```python
from build123d import *

# Parameters (mm, degrees)
BOSS_EXTRUDE1_DEPTH = 32
SKETCH2_R           = 1.75
CUT_EXTRUDE1_DEPTH  = 10
SKETCH3_W           = 67.397349656
SKETCH3_H           = 25.662976956
CUT_EXTRUDE2_DEPTH  = 38.656340887
SKETCH4_R           = 1.75
CUT_EXTRUDE3_DEPTH  = 10


with BuildPart() as part:
    # Sketch1 → Boss-Extrude1 (new body)
    with BuildSketch(Plane(origin=(0, 0, 0), x_dir=(1, 0, 0), z_dir=(0, 1, 0))):
        with BuildLine():
            Line((-8, -10), (-8, -12))
            ThreePointArc((-8, -12), (-8.878679656, -14.121320344), (-11, -15))
            Line((-11, -15), (-13, -15))
            Line((-13, -15), (-13, 15))
            Line((-13, 15), (-1, 15))
            Line((-1, 15), (13, 0))
            Line((13, 0), (13, -15))
            Line((13, -15), (11, -15))
            ThreePointArc((11, -15), (8.878679656, -14.121320344), (8, -12))
            Line((8, -12), (8, -10))
            ThreePointArc((8, -10), (0, -2), (-8, -10))
        make_face()
    extrude(amount=BOSS_EXTRUDE1_DEPTH)

    # Sketch2 → Cut-Extrude1 (cut)
    with BuildSketch(Plane(origin=(13, 0, 0), x_dir=(0, 0, -1), z_dir=(1, 0, 0))):
        with Locations((-10, 26)):
            Circle(SKETCH2_R)
        with Locations((-10, 6)):
            Circle(SKETCH2_R)
    extrude(amount=-CUT_EXTRUDE1_DEPTH, mode=Mode.SUBTRACT)

    # Sketch3 → Cut-Extrude2 (cut, through all)
    with BuildSketch(Plane(origin=(0, 32, 0), x_dir=(1, 0, 0), z_dir=(0, 1, 0))):
        with Locations((-9.275193266, 15.831488478)):
            Rectangle(SKETCH3_W, SKETCH3_H)
    extrude(amount=-CUT_EXTRUDE2_DEPTH, mode=Mode.SUBTRACT)

    # Sketch4 → Cut-Extrude3 (cut)
    with BuildSketch(Plane.ZY.offset(13)):
        with Locations((0, 6)):
            Circle(SKETCH4_R)
        with Locations((0, 26)):
            Circle(SKETCH4_R)
    extrude(amount=-CUT_EXTRUDE3_DEPTH, mode=Mode.SUBTRACT)


solid = part.part
```
Read the model definition and answer for the solid it produces. Units are mm, in the model's axes. A direction names the side the tool comes from. Round coordinates to 2 decimals unless told otherwise and drop trailing zeros. Write each loop counter-clockwise with the first axis right and the second up, starting at its lowest first coordinate (ties: lowest second). Pieces come first, ordered by that corner, then holes. Notation, with made-up numbers: (87.25, 24.25) -> (104.25, 24.25) arc R23 cw to (104.25, 46.25) -> close; hole circle Ø11 at (33.5, -4). An arc over 180 degrees is marked (long way). Answer in a Markdown table with one row per item. Add a question column.
1) Find section B-B, the plane z = 11. Determine the outline of the cut face in (x, y).
2) Find section C-C, the plane y = 15.5. Determine the outline of the cut face in (x, z), and give its area (3 significant figures).
3) Find section A-A, the plane y = 6. Determine the outline of the cut face in (x, z).
4) Which of the six approach directions +Z, -Z, +X, -X, +Y, -Y give full straight-line access (tool end or side, diameter ignored) to faces 1 (the face through (-8.07, 27.735, -0.228)), 2 (the face through (8.9, 15.78, 14.14)), 3 (the face through (10.439, 27.735, 10.228))?
5) Given P1, Ø5, axis at x = 1.5, y = 10.5, coming from the +Z side; P2, Ø3, axis at y = 6, z = 10, coming from the +X side; P3, Ø1, axis at y = 26, z = -1, coming from the -X side, each flat-ended and moving along its own axis, determine where each tip first touches the part or whether it passes through.
6) Determine the mould class of faces 4 (the face through (13, 16, 7)), 5 (the face through (-3, 6, 0)), 6 (the face through (-2, 16, -3)), 7 (the face through (-8, 16, 11)) for opening direction X: pulls with the +X half, pulls with the -X half, needs draft (parallel to the pull), parting line crosses it, or undercut.
7) Find section D-D, the plane x = 0. Determine the outline of the cut face in (y, z), and give its area (3 significant figures).
8) Consider line 1 (Y direction, x = 10.05, z = 10); line 2 (X direction, y = 25.5, z = 11.5); line 3 (Y direction, x = -6.75, z = -1.25). Determine where each line is inside the solid, lowest interval first.
Findings below:
| question | item | result |
|---|---|---|
| 1 | outline | (-13, 0) -> (-8, 0) -> (-8, 32) -> (-13, 32) -> close; (8, 0) -> (13, 0) -> (13, 4.56) -> (8, 4.56) -> close; (8, 7.44) -> (13, 7.44) -> (13, 24.56) -> (8, 24.56) -> close; (8, 27.44) -> (13, 27.44) -> (13, 32) -> (8, 32) -> close |
| 2 | outline | (-13, -3) -> (10.2, -3) -> (13, 0) -> (13, 15) -> (11, 15) arc R3 ccw to (8, 12) -> (8, 10) arc R8 cw to (-8, 10) -> (-8, 12) arc R3 ccw to (-11, 15) -> (-13, 15) -> close |
| 2 | area | 279 mm² |
| 3 | outline | (-13, -3) -> (10.2, -3) -> (13, 0) -> (13, 8.25) -> (7.81, 8.25) arc R8 cw to (-8, 10) -> (-8, 12) arc R3 ccw to (-11, 15) -> (-13, 15) -> (-13, 1.75) -> (-3, 1.75) -> (-3, -1.75) -> (-13, -1.75) -> close; (8, 11.75) -> (13, 11.75) -> (13, 15) -> (11, 15) arc R3 ccw to (8, 12) -> close |
| 4 | face 1 | -X |
| 4 | face 2 | +Z, +Y, -Y |
| 4 | face 3 | +X |
| 5 | P1 | z = 3.07 |
| 5 | P2 | x = -7.86 |
| 5 | P3 | x = -3 |
| 6 | face 4 | pulls with the +X half |
| 6 | face 5 | pulls with the -X half |
| 6 | face 6 | needs draft |
| 6 | face 7 | undercut |
| 7 | outline | (0, -3) -> (32, -3) -> (32, 2) -> (0, 2) -> close |
| 7 | area | 160 mm² |
| 8 | line 1 | 0 to 4.25, 7.75 to 24.25, 27.75 to 32 |
| 8 | line 2 | -13 to -8 |
| 8 | line 3 | 0 to 4.78, 7.22 to 24.78, 27.22 to 32 |
